from build123d import *

# Parameters (mm, degrees)
CROSS_HOLE_SKETCH_R     = 4
CROSS_HOLE_8_DEPTH      = 44
NIPPLE_POCKET_SKETCH_R  = 1.75
NIPPLE_POCKET_3_5_DEPTH = 5
CABLE_BORE_SKETCH_R     = 1.5
CABLE_BORE_3_DEPTH      = 13


with BuildPart() as part:
    # Barrel Profile Sketch → Barrel Body Revolve (revolve)
    with BuildSketch(Plane.XY, mode=Mode.PRIVATE) as barrel_body_revolve_sk:
        Polygon((0, 0), (0, 22), (2.5, 22), (2.5, 14), (6.5, 14), (6.5, 0), align=None)
    revolve(barrel_body_revolve_sk.sketch.rotate(Axis((0, 0, 0), (0, 1, 0)), 90), axis=Axis((0, 0, 0), (0, 1, 0)))

    # Cross Hole Sketch → Cross Hole Ø8 (cut, symmetric)
    with BuildSketch(Plane(origin=(0, 0, 0), x_dir=(0, 0, -1), z_dir=(1, 0, 0))):
        with Locations((0, 7)):
            Circle(CROSS_HOLE_SKETCH_R)
    extrude(amount=CROSS_HOLE_8_DEPTH, both=True, mode=Mode.SUBTRACT)

    # Nipple Pocket Sketch → Nipple Pocket Ø3.5 (cut)
    with BuildSketch(Plane.XZ):
        with Locations(Location((0, 0, 0), (0, 0, 270))):
            Circle(NIPPLE_POCKET_SKETCH_R)
    extrude(amount=-NIPPLE_POCKET_3_5_DEPTH, mode=Mode.SUBTRACT)

    # Cable Bore Sketch → Cable Bore Ø3 (cut)
    with BuildSketch(Plane(origin=(0, 22, 0), x_dir=(1, 0, 0), z_dir=(0, 1, 0))):
        with Locations(Location((0, 0, 0), (0, 0, 270))):
            Circle(CABLE_BORE_SKETCH_R)
    extrude(amount=-CABLE_BORE_3_DEPTH, mode=Mode.SUBTRACT)


solid = part.part
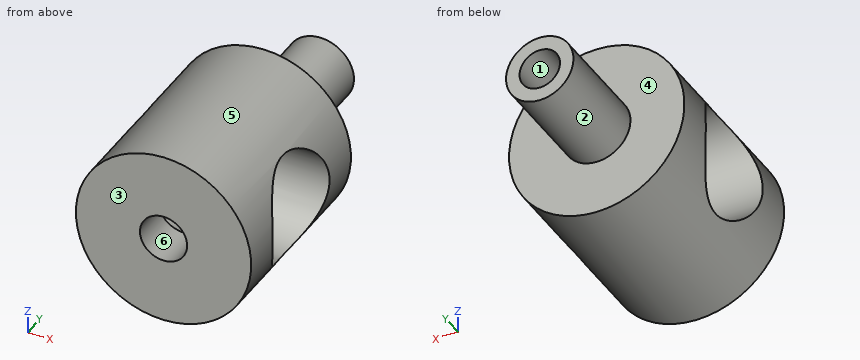
The listing builds one solid part. Answer for the finished solid, in the listing's coordinates (mm). Face numbers are marked on the shaded views. A direction names the side the tool comes from. Coordinates: 2 decimals unless noted, no trailing zeros. Order: outer loops, then holes, each group sorted by start corner. A loop starts at its lowest first (then second) coordinate and runs counter-clockwise, first axis right, second up.
Q1. Consider line 1 (X direction, y = 2.25, z = 0); line 2 (X direction, y = 12.75, z = 0); line 3 (Z direction, x = -1, y = 5.5). Determine where each line is inside the solid, lowest interval first.
Q2. A cutting plane is placed at A-A, the plane x = 0. Write down the section's boundary in (y, z).
Q3. For a pull along Z with two mould halves and no side action, classify the marked faces 1, 2 and 3 as pulls with the +Z half, pulls with the -Z half, needs draft (parallel to the pull), parting line crosses it, or undercut.
Q4. A cutting plane is placed at D-D, the plane y = 16.5. Write down the section's boundary in (x, z).
Q5. Which of the six approach directions +Z, -Z, +X, -X, +Y, -Y give full straight-line access (tool end or side, diameter ignored) to the marked faces 4, 5 and 6?
Q6. A cutting plane is placed at B-B, the plane z = 0. Write down the section's boundary in (x, y).
Q7. A cutting plane is placed at C-C, the plane z = -3.5. Write down the section's boundary in (x, y).
Q8. Given P1, Ø1, axis at y = 11, z = -4.5, coming from the +X side; P2, Ø3, axis at y = 16.5, z = -3.5, coming from the +X side; P3, Ø5, axis at y = 7, z = 0, coming from the -X side (1 decimal); P4, Ø3, axis at x = -4, y = 9, coming from the +Z side, each flat-ended and moving along its own axis, determine where each tip first touches the part or whether it passes through.
Answers follow:
1. line 1: x = -6.5 to -1.75, 1.75 to 6.5
1. line 2: x = -6.5 to -1.5, 1.5 to 6.5
1. line 3: z = -6.42 to -3.71, 3.71 to 6.42
2. outline: (0, -6.5) - (14, -6.5) - (14, -2.5) - (22, -2.5) - (22, -1.5) - (10.71, -1.5) arc R4 cw to (3.4, -1.75) - (0, -1.75) - close; (0, 1.75) - (3.4, 1.75) arc R4 cw to (10.71, 1.5) - (22, 1.5) - (22, 2.5) - (14, 2.5) - (14, 6.5) - (0, 6.5) - close
3. face 1: undercut
3. face 2: parting line crosses it
3. face 3: needs draft
4. outline: circle Ø5 at (0, 0); hole circle Ø3 at (0, 0)
5. face 4: +Y
5. face 5: +Y, -Y
5. face 6: -Y
6. outline: (-6.5, 0) - (-1.75, 0) - (-1.75, 3) - (-6.5, 3) - close; (-6.5, 11) - (-1.5, 11) - (-1.5, 22) - (-2.5, 22) - (-2.5, 14) - (-6.5, 14) - close; (1.5, 11) - (6.5, 11) - (6.5, 14) - (2.5, 14) - (2.5, 22) - (1.5, 22) - close; (1.75, 0) - (6.5, 0) - (6.5, 3) - (1.75, 3) - close
7. outline: (-5.48, 0) - (5.48, 0) - (5.48, 5.06) - (-5.48, 5.06) - close; (-5.48, 8.94) - (5.48, 8.94) - (5.48, 14) - (-5.48, 14) - close
8. P1: stops at x = 5.12
8. P2: stops at x = 1.5
8. P3: passes through
8. P4: stops at z = 6
